Input: part model. Units: mm. Frame: model coordinates. A direction names the side the tool comes from. Coordinates: 2 decimals unless noted, no trailing zeros. Write each loop counter-clockwise with the first axis right and the second up, starting at its lowest first coordinate (ties: lowest second). Pieces come first, ordered by that corner, then holes. Notation, with made-up numbers: (62, 22.5) - (75, 22.5) arc R21 cw to (75, 52.5) - close; hole circle Ø6 at (26, 70.25). An arc over 180 degrees is marked (long way). Use a Markdown table: item, result. Add a question column.
Q1. Section query A-A (x = 198). Return the cut outline in (y, z).
Q2. Mould query, pull axis Y, two halves, no side actions, for faces 6 (the face through (1887, 437, -13)), 7 (the face through (1012, 0, -13)), 8 (the face through (2, 215, -56)), 9 (the face through (1022, 173, 2)). Classes: released by +Y, released by -Y, zero draft, split by the parting line, or undercut.
Q3. Section query C-C (y = 62.5). Return the cut outline in (x, z), then the cut area to 3 significant figures.
Q4. Set-up query: faces 1 (the face through (787, 437, -13)), 2 (the face through (1671, 171, -20)), 3 (the face through (678, 191, -13)), 4 (the face through (2015, 215, -55)), 5 (the face through (1582, 307, -19)). Return all of +Z, -Z, +X, -X, +Y, -Y with unobstructed straight access to the full face (end or side cutting, diameter ignored); none if empty.
Q5. Section query D-D (x = 1473.5). Return the cut outline in (y, z), then the cut area to 3 significant figures.
Q6. Section query B-B (y = 243.5). Return the cut outline in (x, z), then the cut area to 3 significant figures.
Q7. Material intervals for probe 1 along X at (y, z) = (236.5, -19.5); probe 2 along X at (y, z) = (223, -9); probe 3 along X at (y, z) = (359.5, -60.5), sorted ascending. Write a range as from..to.
Q8. Pin query (flat end, axial travel): P1, Ø1.6, axis at x = 467.5, z = -13.5, coming from the -Y side; P2, Ø2, axis at x = 1218.5, y = 0.5, coming from the -Z side. Return the tip coordinate at first contact, or that it passes through.
from build123d import *

# Parameters (mm, degrees)
EXTRUDE_1_DEPTH     = 2
SKETCH_7_W          = 2
SKETCH_7_H          = 437
EXTRUDE_2_DEPTH     = 114
SKETCH_8_W          = 2
SKETCH_8_H          = 437
EXTRUDE_3_DEPTH     = 114
EXTRUDE_4_DEPTH     = 40
SKETCH_10_W         = 1150
SKETCH_10_H         = 200
CUT_EXTRUDE_1_DEPTH = 10
SKETCH_11_W         = 2015
SKETCH_11_H         = 42.467862918
EXTRUDE_5_DEPTH     = 2
SKETCH_12_W         = 1154
SKETCH_12_H         = 204
SKETCH_12_W_2       = 1150
SKETCH_12_H_2       = 200
EXTRUDE_6_DEPTH     = 15
SKETCH_13_W         = 1154
SKETCH_13_H         = 204
SKETCH_13_W_2       = 1130
SKETCH_13_H_2       = 180
EXTRUDE_7_DEPTH     = 2


with BuildPart() as part:
    # 草图2 → 凸台-拉伸1 (new body)
    with BuildSketch(Plane.XY):
        Polygon((1757, 437), (2015, 437), (2015, 0), (0, 0), (0, 437), (1582, 437), (1582, 173), (1757, 173), align=None)
    extrude(amount=EXTRUDE_1_DEPTH)

    # 草图7 → 凸台-拉伸2 (add)
    with BuildSketch(Plane(origin=(0, 0, 0), x_dir=(-1, 0, 0), z_dir=(0, 0, -1))):
        with Locations((-2014, 218.5)):
            Rectangle(SKETCH_7_W, SKETCH_7_H)
    extrude(amount=EXTRUDE_2_DEPTH)

    # 草图8 → 凸台-拉伸3 (add)
    with BuildSketch(Plane(origin=(0, 0, 0), x_dir=(-1, 0, 0), z_dir=(0, 0, -1))):
        with Locations((-1, 218.5)):
            Rectangle(SKETCH_8_W, SKETCH_8_H)
    extrude(amount=EXTRUDE_3_DEPTH)

    # 草图9 → 凸台-拉伸4 (add)
    with BuildSketch(Plane(origin=(0, 0, 0), x_dir=(-1, 0, 0), z_dir=(0, 0, -1))):
        Polygon((-2013, 435), (-1759, 435), (-1759, 171), (-1580, 171), (-1580, 435), (-2, 435), (-2, 437), (-1582, 437), (-1582, 173), (-1757, 173), (-1757, 437), (-2013, 437), align=None)
    extrude(amount=EXTRUDE_4_DEPTH)

    # 草图10 → 切除-拉伸1 (cut)
    with BuildSketch(Plane.XY.offset(2)):
        with Locations((675, 287)):
            Rectangle(SKETCH_10_W, SKETCH_10_H)
    extrude(amount=-CUT_EXTRUDE_1_DEPTH, mode=Mode.SUBTRACT)

    # 草图11 → 凸台-拉伸5 (add)
    with BuildSketch(Plane.XZ):
        with Locations((1007.5, -19.233931459)):
            Rectangle(SKETCH_11_W, SKETCH_11_H)
    extrude(amount=-EXTRUDE_5_DEPTH)

    # 草图12 → 凸台-拉伸6 (add)
    with BuildSketch(Plane(origin=(0, 0, 0), x_dir=(-1, 0, 0), z_dir=(0, 0, -1))):
        with Locations((-675, 287)):
            Rectangle(SKETCH_12_W, SKETCH_12_H)
        with Locations((-675, 287)):
            Rectangle(SKETCH_12_W_2, SKETCH_12_H_2, mode=Mode.SUBTRACT)
    extrude(amount=EXTRUDE_6_DEPTH)

    # 草图13 → 凸台-拉伸7 (add)
    with BuildSketch(Plane(origin=(0, 0, -15), x_dir=(-1, 0, 0), z_dir=(0, 0, -1))):
        with Locations((-675, 287)):
            Rectangle(SKETCH_13_W, SKETCH_13_H)
        with Locations((-675, 287)):
            Rectangle(SKETCH_13_W_2, SKETCH_13_H_2, mode=Mode.SUBTRACT)
    extrude(amount=-EXTRUDE_7_DEPTH)


solid = part.part
Values follow:
| question | item | result |
|---|---|---|
| 1 | outline | (0, -40.47) - (2, -40.47) - (2, 0) - (185, 0) - (185, -15) - (197, -15) - (197, -13) - (187, -13) - (187, 2) - (0, 2) - close; (377, -15) - (389, -15) - (389, 0) - (435, 0) - (435, -40) - (437, -40) - (437, 2) - (387, 2) - (387, -13) - (377, -13) - close |
| 2 | face 6 | released by +Y |
| 2 | face 7 | released by -Y |
| 2 | face 8 | undercut |
| 2 | face 9 | zero draft |
| 3 | outline | (0, -114) - (2, -114) - (2, 0) - (2013, 0) - (2013, -114) - (2015, -114) - (2015, 2) - (0, 2) - close |
| 3 | area | 4,490 mm2 |
| 4 | face 1 | +Z, -Z, +X, -X, +Y |
| 4 | face 2 | -Z |
| 4 | face 3 | +Z |
| 4 | face 4 | +Z, -Z, +X, +Y, -Y |
| 4 | face 5 | +Z, -Z, +Y |
| 5 | outline | (0, -40.47) - (2, -40.47) - (2, 0) - (435, 0) - (435, -40) - (437, -40) - (437, 2) - (0, 2) - close |
| 5 | area | 1,030 mm2 |
| 6 | outline | (0, -114) - (2, -114) - (2, 0) - (98, 0) - (98, -15) - (110, -15) - (110, -13) - (100, -13) - (100, 2) - (0, 2) - close; (1240, -15) - (1252, -15) - (1252, 0) - (1580, 0) - (1580, -40) - (1582, -40) - (1582, 2) - (1250, 2) - (1250, -13) - (1240, -13) - close; (1757, -40) - (1759, -40) - (1759, 0) - (2013, 0) - (2013, -114) - (2015, -114) - (2015, 2) - (1757, 2) - close |
| 6 | area | 2,100 mm2 |
| 7 | probe 1 | 0..2, 1580..1582, 1757..1759, 2013..2015 |
| 7 | probe 2 | 0..2, 98..100, 1250..1252, 1580..1582, 1757..1759, 2013..2015 |
| 7 | probe 3 | 0..2, 2013..2015 |
| 8 | P1 | y = 0 |
| 8 | P2 | z = -40.47 |
